Geometry: final body of the model. Coordinates: model frame, mm. Face numbers are marked on the shaded views. Coordinates: 2 decimals unless noted, no trailing zeros. Write each loop counter-clockwise with the first axis right and the second up, starting at its lowest first coordinate (ties: lowest second). Pieces come first, ordered by that corner, then holes. Notation, with made-up numbers: (26.5, 23.5) - (40.5, 23.5) arc R26 cw to (40.5, 38.5) - close; hole circle Ø6 at (51.25, -14.75). An arc over 180 degrees is marked (long way). Put each result on its own line as item: value.
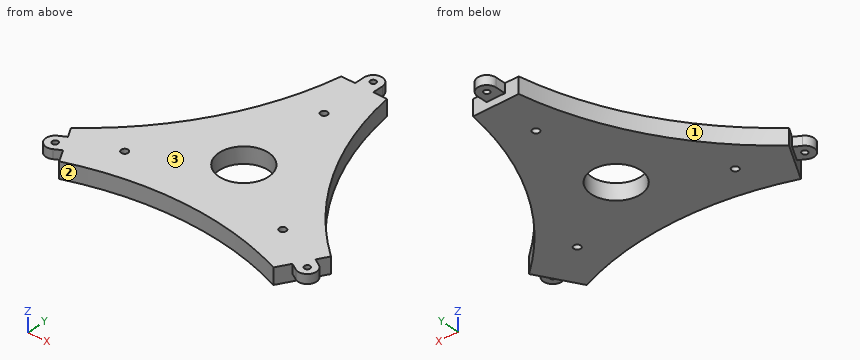
```python
from build123d import *

# Parameters (mm, degrees)
BOSS_EXTRUDE1_DEPTH   = 14
BOSS_EXTRUDE2_DEPTH   = 8
CIRPATTERN1_COUNT     = 3
M6_TAPPED_HOLE1_D     = 5
M6_TAPPED_HOLE1_DEPTH = 15
M6_TAPPED_HOLE1_TIP   = 1.502151548
SKETCH5_R             = 21.5
CUT_EXTRUDE1_DEPTH    = 182.6949343
M6_TAPPED_HOLE2_D     = 5
M6_TAPPED_HOLE2_DEPTH = 15
M6_TAPPED_HOLE2_TIP   = 1.502151548
SKETCH7_R             = 3
CUT_EXTRUDE2_DEPTH    = 17


with BuildPart() as part:
    # Sketch2 → Boss-Extrude1 (new body)
    with BuildSketch(Plane.XY):
        with BuildLine():
            Line((-20, 120), (20, 120))
            ThreePointArc((20, 120), (51.961524227, 30), (113.923048454, -42.679491924))
            Line((113.923048454, -42.679491924), (93.923048454, -77.320508076))
            ThreePointArc((93.923048454, -77.320508076), (0, -60), (-93.923048454, -77.320508076))
            Line((-93.923048454, -77.320508076), (-113.923048454, -42.679491924))
            ThreePointArc((-113.923048454, -42.679491924), (-51.961524227, 30), (-20, 120))
        make_face()
    extrude(amount=BOSS_EXTRUDE1_DEPTH)

    # Sketch3 → Boss-Extrude2 (add)
    with BuildSketch(Plane.XY.offset(14)):
        with BuildLine():
            ThreePointArc((-8, 129), (0, 121), (8, 129))
            Line((8, 129), (-8, 129))
        make_face()
        with BuildLine():
            Line((-8, 129), (8, 129))
            ThreePointArc((8, 129), (0, 137), (-8, 129))
        make_face()
        with BuildLine():
            ThreePointArc((-8, 129), (0, 121), (8, 129))
            Line((8, 129), (-8, 129))
        make_face()
        with BuildLine():
            Line((-8, 129), (8, 129))
            ThreePointArc((8, 129), (0, 137), (-8, 129))
        make_face()
        with BuildLine():
            Line((-8, 120), (8, 120))
            Line((8, 120), (8, 129))
            ThreePointArc((8, 129), (0, 121), (-8, 129))
            Line((-8, 129), (-8, 120))
        make_face()
    boss_extrude2 = extrude(amount=-BOSS_EXTRUDE2_DEPTH)

    # CirPattern1: Boss-Extrude2 ×3 about axis
    cirpattern1_axis = Axis((0, 1.377339071, 0), (0, 0, 1))
    for i in range(1, CIRPATTERN1_COUNT):
        add(boss_extrude2.rotate(cirpattern1_axis, i * 360 / CIRPATTERN1_COUNT))

    # M6 Tapped Hole1
    with Locations(Plane(origin=(0, 129, 6), x_dir=(-1, 0, 0), z_dir=(0, 0, -1))):
        with Locations((0, 0)):
            Hole(M6_TAPPED_HOLE1_D / 2, depth=M6_TAPPED_HOLE1_DEPTH)
            with Locations((0, 0, -(M6_TAPPED_HOLE1_DEPTH + M6_TAPPED_HOLE1_TIP / 2))):  # 118° drill point
                Cone(0, M6_TAPPED_HOLE1_D / 2, M6_TAPPED_HOLE1_TIP, mode=Mode.SUBTRACT)

    # Sketch5 → Cut-Extrude1 (cut, through all)
    with BuildSketch(Plane(origin=(0, 0, 0), x_dir=(-1, 0, 0), z_dir=(0, 0, -1))):
        Circle(SKETCH5_R)
    extrude(amount=-CUT_EXTRUDE1_DEPTH, mode=Mode.SUBTRACT)

    # M6 Tapped Hole2
    with Locations(Plane(origin=(-110.524466463, -62.433991393, 14), x_dir=(1, 0, 0), z_dir=(0, 0, 1))):
        with Locations((0, 0), (221.048932926, 0)):
            Hole(M6_TAPPED_HOLE2_D / 2, depth=M6_TAPPED_HOLE2_DEPTH)
            with Locations((0, 0, -(M6_TAPPED_HOLE2_DEPTH + M6_TAPPED_HOLE2_TIP / 2))):  # 118° drill point
                Cone(0, M6_TAPPED_HOLE2_D / 2, M6_TAPPED_HOLE2_TIP, mode=Mode.SUBTRACT)

    # Sketch7 → Cut-Extrude2 (cut)
    with BuildSketch(Plane(origin=(0, 0, 0), x_dir=(-1, 0, 0), z_dir=(0, 0, -1))):
        with Locations((0, 80)):
            Circle(SKETCH7_R)
        with Locations((69.282032303, -40)):
            Circle(SKETCH7_R)
        with Locations((-69.282032303, -40)):
            Circle(SKETCH7_R)
    extrude(amount=-CUT_EXTRUDE2_DEPTH, mode=Mode.SUBTRACT)


solid = part.part
```
1. Pin query (flat end, axial travel): pin 1 Ø1 at (x, z) = (-82, 4.5) entering from -Y; pin 2 Ø8 at (y, z) = (44, 3) entering from -X; pin 3 Ø6 at (x, z) = (77.5, 12) entering from -Y. Return the tip coordinate at first contact, or that it passes through.
Answer below:
pin 1: stops at y = -73.26
pin 2: stops at x = -46.47
pin 3: stops at y = -72.61
2. Section query B-B (y = 0). Return loops of the section in (x, z).
Answer below:
outline: (-72.15, 0) - (-21.5, 0) - (-21.5, 14) - (-72.15, 14) - close; (21.5, 0) - (72.15, 0) - (72.15, 14) - (21.5, 14) - close
3. Mould query, pull axis X, two halves, no side actions, for the marked faces 1, 2 and 3. Classes: +X half, -X half, draft (parallel to the pull), parting line (faces both ways), or undercut.
Answer below:
face 1: -X half
face 2: undercut
face 3: draft
4. Ray query, probe 1 along Y at (x, z) = (0, 7.75); probe 2 along Y at (x, z) = (4.5, 3.75); probe 3 along X at (y, z) = (18, 7.5). Return the intervals inside material, ascending. Write a range as from..to.
Answer below:
probe 1: y = -60..-21.5, 21.5..77, 83..126.5, 131.5..137
probe 2: y = -60.04..-21.02, 21.02..120
probe 3: x = -59.32..-11.76, 11.76..59.32
5. Section query C-C (x = 12.5). Return loops of the section in (y, z).
Answer below:
outline: (-60.3, 0) - (-17.49, 0) - (-17.49, 14) - (-60.3, 14) - close; (17.49, 0) - (120, 0) - (120, 14) - (17.49, 14) - close
6. Section query A-A (z = 2.5). Return loops of the section in (x, y), then the cut area to 3 significant figures.
Answer below:
outline: (-113.92, -42.68) - (-93.92, -77.32) arc R263.32 cw to (93.92, -77.32) - (113.92, -42.68) arc R263.32 cw to (20, 120) - (-20, 120) arc R263.32 cw to start; hole circle Ø6 at (-69.28, -40); hole circle Ø43 at (0, 0); hole circle Ø6 at (0, 80); hole circle Ø6 at (69.28, -40)
area: 20,900 mm²
7. Section query D-D (y = -40). Return loops of the section in (x, z), then the cut area to 3 significant figures.
Answer below:
outline: (-110.68, 0) - (-72.28, 0) - (-72.28, 14) - (-110.68, 14) - close; (-66.28, 0) - (66.28, 0) - (66.28, 14) - (-66.28, 14) - close; (72.28, 0) - (110.68, 0) - (110.68, 14) - (72.28, 14) - close
area: 2,930 mm²
